Build history of the part. All positions in model axes, mm. A direction names the side the tool comes from. Give positions to 0.01 mm unless a question says otherwise; leave off trailing zeros. Order: outer loops, then holes, each group sorted by start corner. A loop starts at its lowest first (then second) coordinate and runs counter-clockwise, first axis right, second up. Notation, with made-up numbers: M -25,-34 L 6,-34 A30 cw 6,-1 Z; hole C 48,5.5 d7. An arc over 180 degrees is marked long. One line per item, written item: value.
from build123d import *

# Parameters (mm, degrees)
M5_TAPPED_HOLE1_D     = 4.2
M5_TAPPED_HOLE1_DEPTH = 8.4
M5_TAPPED_HOLE1_TIP   = 1.2618073


with BuildPart() as part:
    # Sketch1 → Revolve1 (revolve)
    with BuildSketch(Plane.XY, mode=Mode.PRIVATE) as revolve1_sk:
        Polygon((14, 0), (17.5, 0), (17.5, 25), (22.5, 25), (22.5, 27), (24, 27), (24, 35), (14, 35), align=None)
    revolve(revolve1_sk.sketch.rotate(Axis((0, 0, 0), (0, 1, 0)), 90), axis=Axis((0, 0, 0), (0, 1, 0)))

    # M5 Tapped Hole1
    with Locations(Plane(origin=(0, 35, 0), x_dir=(1, 0, 0), z_dir=(0, 1, 0))):
        with Locations((-19, 0), (19, 0), (13.435028843, 13.435028843), (13.435028843, -13.435028843), (-13.435028843, -13.435028843), (-13.435028843, 13.435028843)):
            Hole(M5_TAPPED_HOLE1_D / 2, depth=M5_TAPPED_HOLE1_DEPTH)
            with Locations((0, 0, -(M5_TAPPED_HOLE1_DEPTH + M5_TAPPED_HOLE1_TIP / 2))):  # 118° drill point
                Cone(0, M5_TAPPED_HOLE1_D / 2, M5_TAPPED_HOLE1_TIP, mode=Mode.SUBTRACT)


solid = part.part
1) Saw through at B-B, the plane y = 30.5. Write the cut outline in (x, z).
Check values:
outline: C 0,0 d48; hole C -19,0 d4.2; hole C -13.44,-13.44 d4.2; hole C -13.44,13.44 d4.2; hole C 0,0 d28; hole C 13.44,-13.44 d4.2; hole C 13.44,13.44 d4.2; hole C 19,0 d4.2
2) Tool access for faces 4 (the face through (-21.003, 30.741, -0.631)), 5 (the face through (12.4, 17.3, -6.5)), 6 (the face through (17.084, 12.675, 3.794)): list every direction of +Z, -Z, +X, -X, +Y, -Y with a clear straight run to the whole face (end or side of a thin tool).
Check values:
face 4: +Y
face 5: +Y, -Y
face 6: -Y
3) Pin check, flat tips, straight feed: pin 1 (5.5 mm diameter, centred on x = -13.44, z = -13.44, fed in from -Y); pin 2 (5 mm diameter, centred on x = 17.5, z = -15, fed in from -Y); pin 3 (2 mm diameter, centred on x = -19, y = 23.5, fed in from -Z); pin 4 (3.5 mm diameter, centred on x = 13.44, z = -13.44, fed in from +Y). Stop position of each tip, or through.
Check values:
pin 1: y = 0
pin 2: y = 25
pin 3: through
pin 4: y = 26.39
4) Saw through at D-D, the plane y = 20. Write the cut outline in (x, z), then the cut area to 3 significant figures.
Check values:
outline: C 0,0 d35; hole C 0,0 d28
area: 346 mm^2
5) Mould opens along Z. For faces 1 (the face through (13, 25, 12)), 2 (the face through (-7.21, 31.06, -22.89)), 3 (the face through (18.636, 25.557, -0.016)) say: released by +Z, released by -Z, zero draft, split by the parting line, or undercut.
Check values:
face 1: zero draft
face 2: split by the parting line
face 3: undercut
6) Saw through at C-C, the plane z = 4.5. Write the cut outline in (x, y).
Check values:
outline: M -23.57,27 L -22.05,27 L -22.05,25 L -16.91,25 L -16.91,0 L -13.26,0 L -13.26,35 L -23.57,35 Z; M 13.26,0 L 16.91,0 L 16.91,25 L 22.05,25 L 22.05,27 L 23.57,27 L 23.57,35 L 13.26,35 Z
7) Drill centre lines: probe 1 along Z at (x, y) = (-0.5, 26); probe 2 along X at (y, z) = (11, 0); probe 3 along Z at (x, y) = (2, 15). Where is each one in solid material? Low to high. Write a range as from..to.
Check values:
probe 1: -22.49..-13.99, 13.99..22.49
probe 2: -17.5..-14, 14..17.5
probe 3: -17.39..-13.86, 13.86..17.39
8) Saw through at A-A, the plane x = 0. Write the cut outline in (y, z), then the cut area to 3 significant figures.
Check values:
outline: M 0,-17.5 L 25,-17.5 L 25,-22.5 L 27,-22.5 L 27,-24 L 35,-24 L 35,-14 L 0,-14 Z; M 0,14 L 35,14 L 35,24 L 27,24 L 27,22.5 L 25,22.5 L 25,17.5 L 0,17.5 Z
area: 369 mm^2
